For this review, use the dimensioned drawing (mm, ordinates from the lowest corner) and the shaded views. Coordinates: 2 decimals unless noted, no trailing zeros. Write each loop counter-clockwise with the first axis right and the second up, starting at its lowest first coordinate (ties: lowest second). Pieces come first, ordered by that corner, then holes. Notation, with made-up numbers: (-5.75, 27) - (31.25, 27) arc R30 ccw to (31.25, 60) - close; hole circle Ø8 at (-38.5, 54.5). An arc over 180 degrees is marked (long way). One line per item, written item: value.
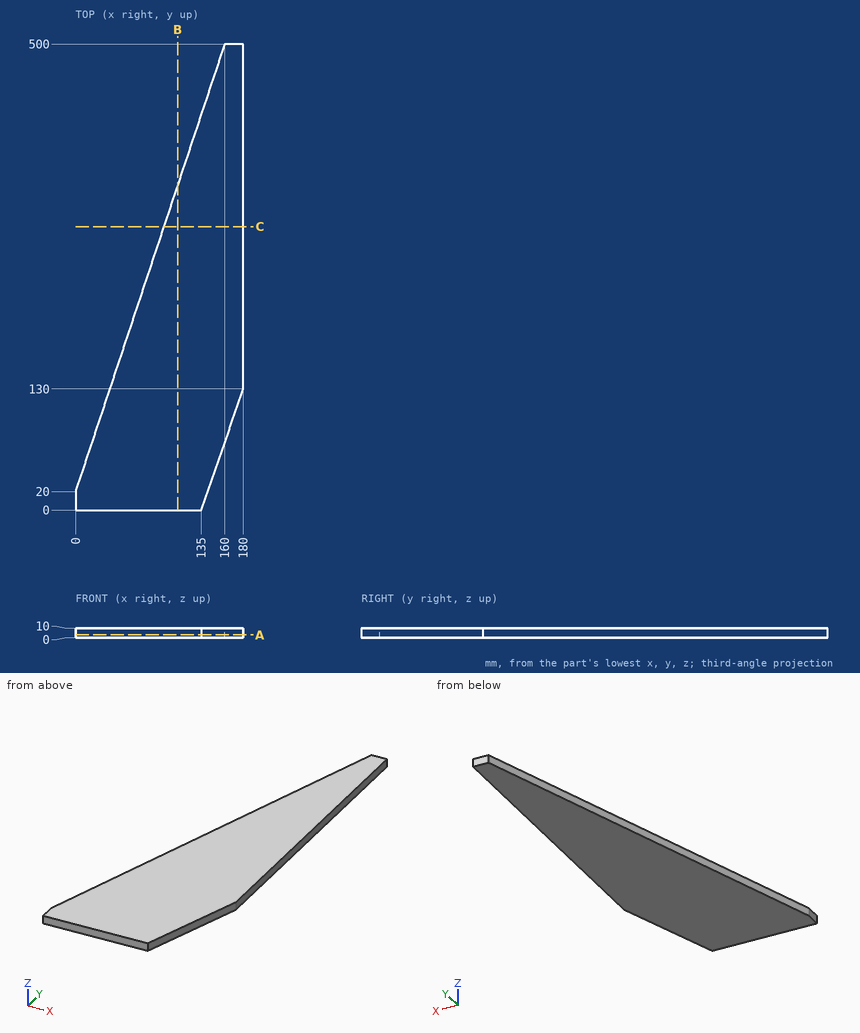
1. Consider section B-B, the plane x = 109.5. Write out the cut boundary in (y, z).
Answer block:
outline: (0, 0) - (348.5, 0) - (348.5, 10) - (0, 10) - close
2. Insertion check: pin 1 Ø6 at (x, z) = (119.5, 2.5) entering from -Y. The pin has a flat end and moves straight along its axis. Give the tip position at first contact, or say it passes through.
Answer block:
pin 1: stops at y = 0
3. Consider section A-A, the plane z = 2.75. Write out the cut boundary in (x, y).
Answer block:
outline: (0, 0) - (135, 0) - (180, 130) - (180, 500) - (160, 500) - (0, 20) - close
4. Wall thickness on line 1 along X through (y, z) = (247.5, 0.75); line 2 along X through (y, z) = (373, 1.25): over which ranges is each line inside the solid? List them lowest first.
Answer block:
line 1: x = 75.83 to 180
line 2: x = 117.67 to 180
5. Consider section C-C, the plane y = 304. Write out the cut boundary in (x, z), then the cut area to 3 significant figures.
Answer block:
outline: (94.67, 0) - (180, 0) - (180, 10) - (94.67, 10) - close
area: 853 mm^2
